Input: part model. Units: mm. Frame: model coordinates. A direction names the side the tool comes from. Round coordinates to 2 decimals unless told otherwise and drop trailing zeros. Loops run counter-clockwise (first coordinate to the right, second up) from the corner with the lowest first, then second, coordinate; pieces in that order, holes last. Notation, with made-up numbers: (8, -1) -> (15, -1) arc R17 cw to (15, 21) -> close; hole circle Ø11 at (81.5, 44). An arc over 180 degrees is marked (long way). Answer as a JSON object with one key per item and string values. Group by question number.
Item 1: Set-up query: faces 4 (the flat face through (50, 60, 11)), 5 (the cylindrical face through (43.97, 57.596, 24.565)), 6 (the flat face through (-5, 22.25, 15)). Return all of +Z, -Z, +X, -X, +Y, -Y with unobstructed straight access to the full face (end or side cutting, diameter ignored); none if empty.
Item 2: Draft query along Z for faces 1 (the conical face through (42.758, 61.423, 18.585)), 2 (the flat face through (-5, 39, 1)), 3 (the cylindrical face through (43.635, 6.449, 18.71)). Return one class per face: released by +Z, released by -Z, zero draft, split by the parting line, or undercut.
Item 3: Section query C-C on x = 10.5. Return loops of the section in (y, z), and give its area (3 significant figures).
Item 4: Section query B-B on z = 6. Return loops of the section in (x, y), and give its area (3 significant figures).
Item 5: Section query A-A on y = 25. Return loops of the section in (x, z), and give its area (3 significant figures).
Item 6: Material intervals for line 1 (Z direction, x = 49.5, y = 70.5); line 2 (X direction, y = 28, z = 15); line 3 (Y direction, x = -5, z = 21), sorted ascending. Write a range as [from, to].
Item 7: Pin query (flat end, axial travel): pin 1 (11.5 mm diameter, centred on x = 46, y = 61.5, fed in from +Z); pin 2 (4 mm diameter, centred on x = 5.5, z = 4.5, fed in from +Y); pin 3 (3 mm diameter, centred on x = -3.5, z = 13.5, fed in from +Y); pin 4 (1.8 mm diameter, centred on x = 45.5, y = 62, fed in from +Z). Return the tip coordinate at first contact, or that it passes through.
from build123d import *

# Parameters (mm, degrees)
BOSS_EXTRUDE1_DEPTH     = 30
SKETCH2_R               = 1
CUT_EXTRUDE1_DEPTH      = 25
SKETCH3_R               = 3
CUT_EXTRUDE2_DEPTH      = 28
SKETCH4_R               = 3
CUT_EXTRUDE3_DEPTH      = 61.5
CUT_EXTRUDE4_DEPTH      = 20
CHAMFER1_SIZE           = 2
G1_8_TAPPED_HOLE1_D     = 8.8
G1_8_TAPPED_HOLE1_DEPTH = 12.72
G1_8_TAPPED_HOLE1_TIP   = 2.643786724
G1_8_TAPPED_HOLE2_D     = 8.8
G1_8_TAPPED_HOLE2_DEPTH = 10.72
G1_8_TAPPED_HOLE2_TIP   = 2.643786724


with BuildPart() as part:
    # Sketch1 → Boss-Extrude1 (new body)
    with BuildSketch(Plane.XY):
        Polygon((-10, 40), (-10, 0), (52.5, 0), (52.5, 85), (40.5, 85), (40.5, 15), (0, 15), (0, 40), align=None)
    extrude(amount=BOSS_EXTRUDE1_DEPTH)

    # Sketch2 → Cut-Extrude1 (cut)
    with BuildSketch(Plane(origin=(0, 85, 0), x_dir=(1, 0, 0), z_dir=(0, 1, 0))):
        with Locations(Location((49.5, -3, 0), (0, 0, 270))):
            Circle(SKETCH2_R)
        with Locations(Location((49.5, -11, 0), (0, 0, 270))):
            Circle(SKETCH2_R)
        with Locations(Location((49.5, -19, 0), (0, 0, 270))):
            Circle(SKETCH2_R)
    extrude(amount=-CUT_EXTRUDE1_DEPTH, mode=Mode.SUBTRACT)

    # Sketch3 → Cut-Extrude2 (cut)
    with BuildSketch(Plane.XY.offset(30)):
        with Locations((46, 61.5)):
            Circle(SKETCH3_R)
    extrude(amount=-CUT_EXTRUDE2_DEPTH, mode=Mode.SUBTRACT)

    # Sketch4 → Cut-Extrude3 (cut)
    with BuildSketch(Plane.XZ):
        with Locations(Location((46, 15, 0), (0, 0, 270))):
            Circle(SKETCH4_R)
    extrude(amount=-CUT_EXTRUDE3_DEPTH, mode=Mode.SUBTRACT)

    # Sketch5 → Cut-Extrude4 (cut)
    with BuildSketch(Plane.ZY.offset(10)):
        with BuildLine():
            Line((7.5, 27.75), (22.5, 27.75))
            ThreePointArc((22.5, 27.75), (25.25, 25), (22.5, 22.25))
            Line((22.5, 22.25), (7.5, 22.25))
            ThreePointArc((7.5, 22.25), (4.75, 25), (7.5, 27.75))
        make_face()
    extrude(amount=-CUT_EXTRUDE4_DEPTH, mode=Mode.SUBTRACT)

    # Chamfer1
    chamfer1_edges = [part.edges().sort_by_distance(p)[0] for p in [
        (-5, 40, 0),
        (-10, 0, 15),
        (-5, 40, 30),
    ]]
    chamfer(chamfer1_edges, length=CHAMFER1_SIZE)

    # G1/8 Tapped Hole1
    with Locations(Plane.XZ):
        with Locations((46, 15)):
            Hole(G1_8_TAPPED_HOLE1_D / 2, depth=G1_8_TAPPED_HOLE1_DEPTH)
            with Locations((0, 0, -(G1_8_TAPPED_HOLE1_DEPTH + G1_8_TAPPED_HOLE1_TIP / 2))):  # 118° drill point
                Cone(0, G1_8_TAPPED_HOLE1_D / 2, G1_8_TAPPED_HOLE1_TIP, mode=Mode.SUBTRACT)

    # G1/8 Tapped Hole2
    with Locations(Plane.XY.offset(30)):
        with Locations((46, 61.5)):
            Hole(G1_8_TAPPED_HOLE2_D / 2, depth=G1_8_TAPPED_HOLE2_DEPTH)
            with Locations((0, 0, -(G1_8_TAPPED_HOLE2_DEPTH + G1_8_TAPPED_HOLE2_TIP / 2))):  # 118° drill point
                Cone(0, G1_8_TAPPED_HOLE2_D / 2, G1_8_TAPPED_HOLE2_TIP, mode=Mode.SUBTRACT)


solid = part.part
Solved:
{
 "1": {"face 4": "+Y", "face 5": "+Z", "face 6": "-X"},
 "2": {"face 1": "released by +Z", "face 2": "released by -Z", "face 3": "undercut"},
 "3": {"outline": "(0, 0) -> (15, 0) -> (15, 30) -> (0, 30) -> close", "area": "450 mm²"},
 "4": {"outline": "(-10, 2) -> (-8, 0) -> (52.5, 0) -> (52.5, 85) -> (40.5, 85) -> (40.5, 15) -> (0, 15) -> (0, 22.7) -> (-10, 22.7) -> close; (-10, 27.3) -> (0, 27.3) -> (0, 40) -> (-10, 40) -> close; hole circle Ø6 at (46, 61.5)", "area": "1,950 mm²"},
 "5": {"outline": "(-10, 0) -> (0, 0) -> (0, 4.75) -> (-10, 4.75) -> close; (-10, 25.25) -> (0, 25.25) -> (0, 30) -> (-10, 30) -> close; (40.5, 0) -> (52.5, 0) -> (52.5, 30) -> (40.5, 30) -> close; hole circle Ø6 at (46, 15)", "area": "427 mm²"},
 "6": {"line 1": "[0, 2], [4, 10], [12, 18], [20, 30]", "line 2": "[-10, 0], [40.5, 43], [49, 52.5]", "line 3": "[0, 22.25], [27.75, 40]"},
 "7": {"pin 1": "z = 30", "pin 2": "y = 15", "pin 3": "y = 40", "pin 4": "z = 2"}
}
